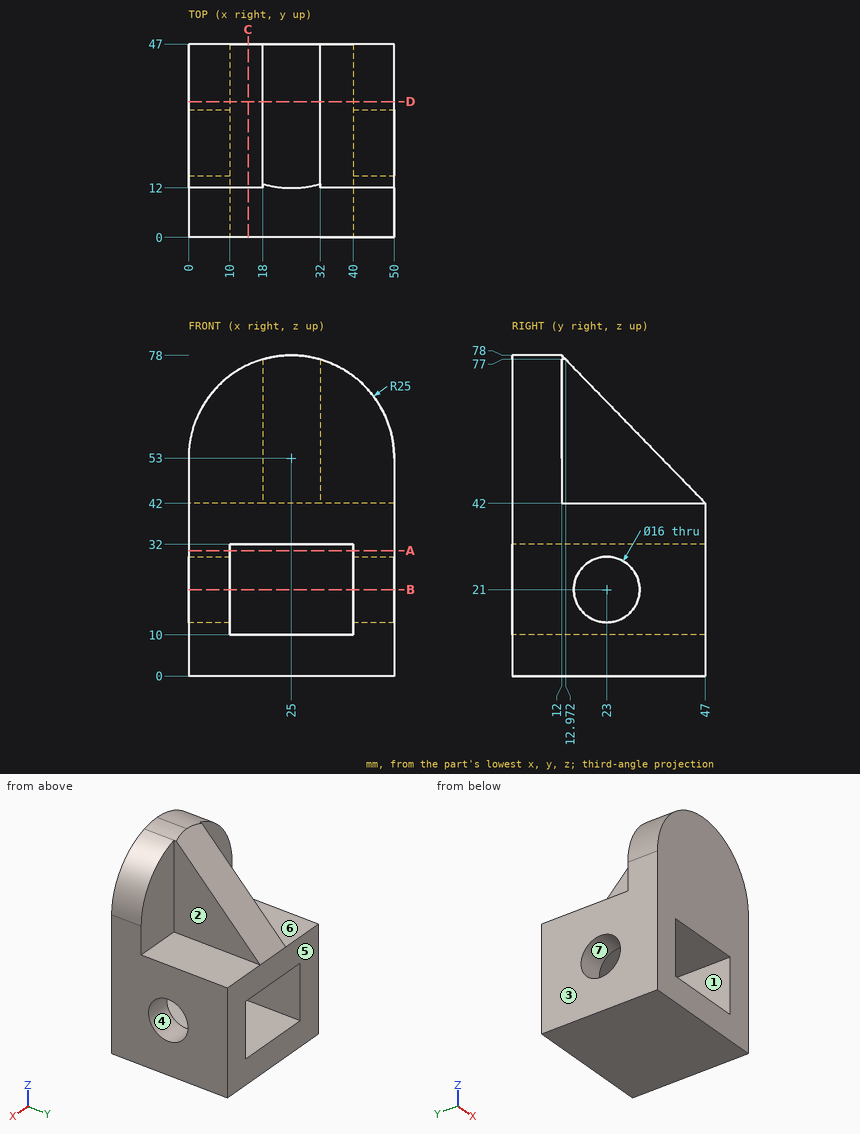
Geometry check sheet. Reference: drawing and pictorial views, mm from the part's lowest x, y, z. A direction names the side the tool comes from. Round coordinates to 2 decimals unless told otherwise and drop trailing zeros. Loops run counter-clockwise (first coordinate to the right, second up) from the corner with the lowest first, then second, coordinate; pieces in that order, holes last. Notation, with made-up numbers: (-34, -18.75) -> (-21, -18.75) arc R25 ccw to (-21, 17.25) -> close; hole circle Ø8 at (1, 68). An arc over 180 degrees is marked (long way). Use a Markdown table: item, result.
(1) Set-up check for the marked faces 1, 2 and 3: record each of +Z, -Z, +X, -X, +Y, -Y from which the full face is reachable in a straight line by a thin tool's end or side.
Calculated:
| item | result |
|---|---|
| face 1 | +Y, -Y |
| face 2 | +Z, +X, +Y |
| face 3 | +Z, -Z, -X, +Y, -Y |
(2) Go/stop test with flat-tipped pins: P1, Ø8, axis at x = 36.5, y = 13, coming from the +Z side; P2, Ø9.5, axis at y = 23, z = 21, coming from the +X side; P3, Ø12, axis at y = 29, z = 55.5, coming from the +X side; P4, Ø1, axis at x = 15, y = 35.5, coming from the -Z side. Record where each tip stops, or that it passes through.
Calculated:
| item | result |
|---|---|
| P1 | z = 76.81 |
| P2 | through |
| P3 | x = 32 |
| P4 | z = 0 |
(3) Mould release check, pull along Y, two halves, no side actions. Record for the marked faces 4, 5, 6 and 7: released by +Y, released by -Y, zero draft, split by the parting line, or undercut.
Calculated:
| item | result |
|---|---|
| face 4 | undercut |
| face 5 | released by +Y |
| face 6 | zero draft |
| face 7 | undercut |
(4) Sectioned sample at C-C (x = 14.5). Enter the section's corners in (y, z), then the cut area to 3 significant figures.
Calculated:
| item | result |
|---|---|
| outline | (0, 0) -> (47, 0) -> (47, 10) -> (0, 10) -> close; (0, 32) -> (47, 32) -> (47, 42) -> (12, 42) -> (12, 75.69) -> (0, 75.69) -> close |
| area | 1,340 mm² |
(5) Sectioned sample at D-D (y = 33). Enter the section's corners in (x, z).
Calculated:
| item | result |
|---|---|
| outline | (0, 0) -> (50, 0) -> (50, 42) -> (32, 42) -> (32, 56.4) -> (18, 56.4) -> (18, 42) -> (0, 42) -> close; hole (10, 10) -> (40, 10) -> (40, 32) -> (10, 32) -> close |
(6) Sectioned sample at A-A (z = 30.5). Enter the section's corners in (x, y).
Calculated:
| item | result |
|---|---|
| outline | (0, 0) -> (10, 0) -> (10, 47) -> (0, 47) -> close; (40, 0) -> (50, 0) -> (50, 47) -> (40, 47) -> close |
(7) Sectioned sample at B-B (z = 21). Enter the section's corners in (x, y).
Calculated:
| item | result |
|---|---|
| outline | (0, 0) -> (10, 0) -> (10, 15) -> (0, 15) -> close; (0, 31) -> (10, 31) -> (10, 47) -> (0, 47) -> close; (40, 0) -> (50, 0) -> (50, 15) -> (40, 15) -> close; (40, 31) -> (50, 31) -> (50, 47) -> (40, 47) -> close |
(8) Scan lines: probe 1 along Z at (x, y) = (37, 23); probe 2 along X at (y, z) = (11, 16.5); probe 3 along Y at (x, z) = (7, 21). Record each from-to range of solid material in increasing order.
Calculated:
| item | result |
|---|---|
| probe 1 | 0 to 10, 32 to 42 |
| probe 2 | 0 to 10, 40 to 50 |
| probe 3 | 0 to 15, 31 to 47 |
